from build123d import *

# Parameters (mm, degrees)
EXTRUDE_1_DEPTH = 50
CHAMFER_1_SIZE  = 3


with BuildPart() as part:
    # 草图2 → 凸台-拉伸1 (new, symmetric)
    with BuildSketch(Plane(origin=(409.637600706, 0.5, -34.379468655), x_dir=(1, 0, 0), z_dir=(0, 0, 1))):
        Polygon((-409.637600706, 92.5), (-409.637600706, -0.5), (-457.637600706, -0.5), (-457.637600706, 7.5), (-417.637600706, 7.5), (-417.637600706, 92.5), align=None)
    extrude(amount=EXTRUDE_1_DEPTH, both=True)

    # 倒角1
    chamfer_1_edges = [part.edges().sort_by_distance(p)[0] for p in [
        (-48, 4, 15.620531345),
        (-4, 93, 15.620531345),
        (-48, 4, -84.379468655),
        (-4, 93, -84.379468655),
    ]]
    chamfer(chamfer_1_edges, length=CHAMFER_1_SIZE)


solid = part.part
The model under review builds one solid part; all positions refer to its coordinate system, in mm. A direction names the side the tool comes from. Give positions to 0.01 mm unless a question says otherwise; leave off trailing zeros. Loops run counter-clockwise (first coordinate to the right, second up) from the corner with the lowest first, then second, coordinate; pieces in that order, holes last. Notation, with made-up numbers: (0.5, -11.75) -> (7.5, -11.75) arc R30 ccw to (7.5, 22.25) -> close; hole circle Ø2 at (75, -2.75). An arc over 180 degrees is marked (long way). Answer as a JSON object with one key per item and string values. Group by question number.
Q1. Take a section at A-A (z = -29). Write out the cut boundary in (x, y), plus the area to 3 significant figures.
Q2. Wall thickness on line 1 along X through (y, z) = (16, -70); line 2 along Y through (x, z) = (-18, -53): over which ranges is each line inside the solid? List them lowest first.
Q3. Tool access review of faces 1 (the flat face through (-8, 50, -34)), 2 (the flat face through (-4.06, 91.52, 14.1)): name each direction out of +Z, -Z, +X, -X, +Y, -Y from which nothing blocks a thin tool from reaching the whole face with its end or side.
Q4. Take a section at C-C (x = -28). Write out the cut boundary in (y, z).
Q5. Take a section at B-B (y = 73.5). Write out the cut boundary in (x, z).
Q6. Insertion check: pin 1 (5 mm diameter, centred on y = 70.5, z = -59.5, fed in from -X); pin 2 (10 mm diameter, centred on y = 75, z = -63, fed in from +X); pin 3 (12 mm diameter, centred on x = -23, z = -50, fed in from +Y). Each pin has a flat end and moves straight along its axis. Give the tip position at first contact, or say it passes through.
Answer below:
{
 "1": {"outline": "(-48, 0) -> (0, 0) -> (0, 93) -> (-8, 93) -> (-8, 8) -> (-48, 8) -> close", "area": "1,060 mm2"},
 "2": {"line 1": "x = -8 to 0", "line 2": "y = 0 to 8"},
 "3": {"face 1": "+Z, -Z, -X, +Y", "face 2": "+Z, +X, -X, +Y"},
 "4": {"outline": "(0, -84.38) -> (8, -84.38) -> (8, 15.62) -> (0, 15.62) -> close"},
 "5": {"outline": "(-8, -84.38) -> (0, -84.38) -> (0, 15.62) -> (-8, 15.62) -> close"},
 "6": {"pin 1": "stops at x = -8", "pin 2": "stops at x = 0", "pin 3": "stops at y = 8"}
}
